```python
from build123d import *

# Parameters (mm, degrees)
BASE_FLANGE_DEPTH        = 5
CLAMP_BODY_DEPTH         = 20
BORE_28_DEPTH            = 20
FLANGE_CUT_SKETCH_R      = 5
FLANGE_CUT_DEPTH         = 20
LUG_A_DEPTH              = 5
LUG_A_WEB_SKETCH_W       = 5
LUG_A_WEB_SKETCH_H       = 10
LUG_A_WEB_DEPTH          = 7
LUG_B_DEPTH              = 5
LUG_BRIDGE_SKETCH_W      = 5
LUG_BRIDGE_SKETCH_H      = 10
LUG_BRIDGE_DEPTH         = 7
EAR_A_DEPTH              = 7
EAR_START                = -7
EAR_B_DEPTH              = 7
CLAMP_BOLT_HOLE_SKETCH_R = 3
CLAMP_BOLT_HOLE_6_DEPTH  = 70


with BuildPart() as part:
    # Base Flange Sketch → Base Flange (new body)
    with BuildSketch(Plane.XY):
        with BuildLine():
            Line((62, -10), (0, -10))
            ThreePointArc((0, -10), (-10, 0), (0, 10))
            Line((0, 10), (62, 10))
            ThreePointArc((62, 10), (72, 0), (62, -10))
        make_face()
    extrude(amount=BASE_FLANGE_DEPTH)

    # Clamp Body Sketch → Clamp Body (add)
    with BuildSketch(Plane.XZ.offset(10)):
        with BuildLine():
            Line((10, 5), (52, 5))
            Line((52, 5), (52, 20))
            ThreePointArc((52, 20), (31, 41), (10, 20))
            Line((10, 20), (10, 5))
        make_face()
    extrude(amount=-CLAMP_BODY_DEPTH)

    # Bore Sketch → Bore Ø28 (cut)
    with BuildSketch(Plane.XZ.offset(10)):
        with BuildLine():
            Line((17, 5), (17, 20))
            ThreePointArc((17, 20), (31, 34), (45, 20))
            Line((45, 20), (45, 5))
            Line((45, 5), (17, 5))
        make_face()
    extrude(amount=-BORE_28_DEPTH, mode=Mode.SUBTRACT)

    # Flange Cut Sketch → Flange Cut (cut)
    with BuildSketch(Plane.XY.offset(5)):
        with Locations((62, 0)):
            Circle(FLANGE_CUT_SKETCH_R)
        Circle(FLANGE_CUT_SKETCH_R)
    extrude(amount=-FLANGE_CUT_DEPTH, mode=Mode.SUBTRACT)

    # Lug A Sketch → Lug A (add)
    with BuildSketch(Plane.XY.offset(5)):
        with BuildLine():
            Line((10, -10), (5, -10))
            ThreePointArc((5, -10), (8.535533906, -11.464466094), (10, -15))
            Line((10, -15), (10, -20))
            Line((10, -20), (17, -20))
            Line((17, -20), (17, -10))
            Line((17, -10), (10, -10))
        make_face()
    extrude(amount=-LUG_A_DEPTH)

    # Lug A Web Sketch → Lug A Web (add)
    with BuildSketch(Plane(origin=(17, 0, 0), x_dir=(0, 0, -1), z_dir=(1, 0, 0))):
        with Locations((-7.5, -15)):
            Rectangle(LUG_A_WEB_SKETCH_W, LUG_A_WEB_SKETCH_H)
    extrude(amount=-LUG_A_WEB_DEPTH)

    # Lug B Sketch → Lug B (add)
    with BuildSketch(Plane.XY.offset(5)):
        with BuildLine():
            Line((52, -10), (57, -10))
            ThreePointArc((57, -10), (53.464466094, -11.464466094), (52, -15))
            Line((52, -15), (52, -20))
            Line((52, -20), (45, -20))
            Line((45, -20), (45, -10))
            Line((45, -10), (52, -10))
        make_face()
    extrude(amount=-LUG_B_DEPTH)

    # Lug Bridge Sketch → Lug Bridge (add)
    with BuildSketch(Plane.ZY.offset(-45)):
        with Locations((7.5, -15)):
            Rectangle(LUG_BRIDGE_SKETCH_W, LUG_BRIDGE_SKETCH_H)
    extrude(amount=-LUG_BRIDGE_DEPTH)

    # Ear A Sketch → Ear A (add)
    with BuildSketch(Plane.ZY.offset(-10)):
        with BuildLine():
            Line((0, -20), (10, -20))
            ThreePointArc((10, -20), (5, -25), (0, -20))
        make_face()
    extrude(amount=-EAR_A_DEPTH)

    # Ear B Sketch → Ear B (add)
    with BuildSketch(Plane(origin=(52, 0, 0), x_dir=(0, 0, -1), z_dir=(1, 0, 0)).offset(EAR_START)):
        with BuildLine():
            Line((-10, -20), (0, -20))
            ThreePointArc((0, -20), (-5, -25), (-10, -20))
        make_face()
    extrude(amount=EAR_B_DEPTH)

    # Clamp Bolt Hole Sketch → Clamp Bolt Hole Ø6 (cut)
    with BuildSketch(Plane(origin=(52, 0, 0), x_dir=(0, 0, -1), z_dir=(1, 0, 0))):
        with Locations(Location((-5, -20, 0), (0, 0, 90))):
            Circle(CLAMP_BOLT_HOLE_SKETCH_R)
    extrude(amount=-CLAMP_BOLT_HOLE_6_DEPTH, mode=Mode.SUBTRACT)


solid = part.part
```
Check sheet for the modelled part. Datum: model origin and axes. Units: mm. A direction names the side the tool comes from. Coordinates: 2 decimals unless noted, no trailing zeros. Write each loop counter-clockwise with the first axis right and the second up, starting at its lowest first coordinate (ties: lowest second). Pieces come first, ordered by that corner, then holes. Notation, with made-up numbers: M 9.5,62 L 47.5,62 A20 ccw 47.5,74 Z; hole C 13.25,73.5 d4. An arc over 180 degrees is marked long. Write item = value, one per line. Start each with the question number.
1. Sectioned sample at C-C (z = 3.5). Record the cut outline in (x, y), then the cut area to 3 significant figures.
2. Sectioned sample at B-B (y = -11). Record the cut outline in (x, z).
3. Thickness scan on probe 1 along X at (y, z) = (-5.5, 13.5); probe 2 along Z at (x, y) = (48, -20); probe 3 along X at (y, z) = (-2, 32). Record the ranges inside material, lowest first.
4. Tool access check on faces 4 (the flat face through (60, -10, 2)), 5 (the cylindrical face through (31, 0, 34)), 6 (the flat face through (3, -10, 2)). Record the directions out of +Z, -Z, +X, -X, +Y, -Y that give a thin tool (end or side, any length) a straight path to the whole face; none if there is none.
5. Sectioned sample at D-D (x = 31). Record the cut outline in (y, z), then the cut area to 3 significant figures.
6. Mould release check, pull along Y, two halves, no side actions. Record for faces 1 (the flat face through (57.7, 3.2, 5)), 2 (the cylindrical face through (48.5, -22.4, 3.2)), 3 (the cylindrical face through (72, 0, 2)): pulls with the +Y half, pulls with the -Y half, needs draft (parallel to the pull), parting line crosses it, or undercut.
7. Sectioned sample at A-A (y = 0). Record the cut outline in (x, z).
8. Go/stop test with flat-tipped pins: pin 1 (2.5 mm diameter, centred on x = 60.5, z = 3.5, fed in from -Y); pin 2 (10 mm diameter, centred on x = 32.5, y = -3.5, fed in from +Z); pin 3 (3.5 mm diameter, centred on x = 48, y = -14, fed in from +Z). Record where each tip stops, or that it passes through.
The answers:
q1.outline = M 0,-10 L 5,-10 A5 cw 10,-15 L 10,-17.4 L 17,-17.4 L 17,-10 L 45,-10 L 45,-17.4 L 52,-17.4 L 52,-15 A5 cw 57,-10 L 62,-10 A10 ccw 62,10 L 0,10 A10 ccw Z; M 10,-24.77 L 17,-24.77 L 17,-22.6 L 10,-22.6 Z; M 45,-24.77 L 52,-24.77 L 52,-22.6 L 45,-22.6 Z; hole C 0,0 d10; hole C 62,0 d10
q1.area = 1,540 mm²
q2.outline = M 8,0 L 17,0 L 17,10 L 10,10 L 10,5 L 8,5 Z; M 45,0 L 54,0 L 54,5 L 52,5 L 52,10 L 45,10 Z
q3.probe_1 = 10 to 17, 45 to 52
q3.probe_2 = 0 to 2, 8 to 10
q3.probe_3 = 13.77 to 23.79, 38.21 to 48.23
q4.face_4 = +Z, -Z, +X, -Y
q4.face_5 = +Y, -Y
q4.face_6 = +Z, -Z, -X, -Y
q5.outline = M -10,0 L 10,0 L 10,5 L -10,5 Z; M -10,34 L 10,34 L 10,41 L -10,41 Z
q5.area = 240 mm²
q6.face_1 = needs draft
q6.face_2 = undercut
q6.face_3 = parting line crosses it
q7.outline = M -10,0 L -5,0 L -5,5 L -10,5 Z; M 5,0 L 57,0 L 57,5 L 52,5 L 52,20 A21 ccw 10,20 L 10,5 L 5,5 Z; M 67,0 L 72,0 L 72,5 L 67,5 Z; hole M 17,5 L 45,5 L 45,20 A14 ccw 17,20 Z
q8.pin_1 = -10
q8.pin_2 = 41
q8.pin_3 = 10
